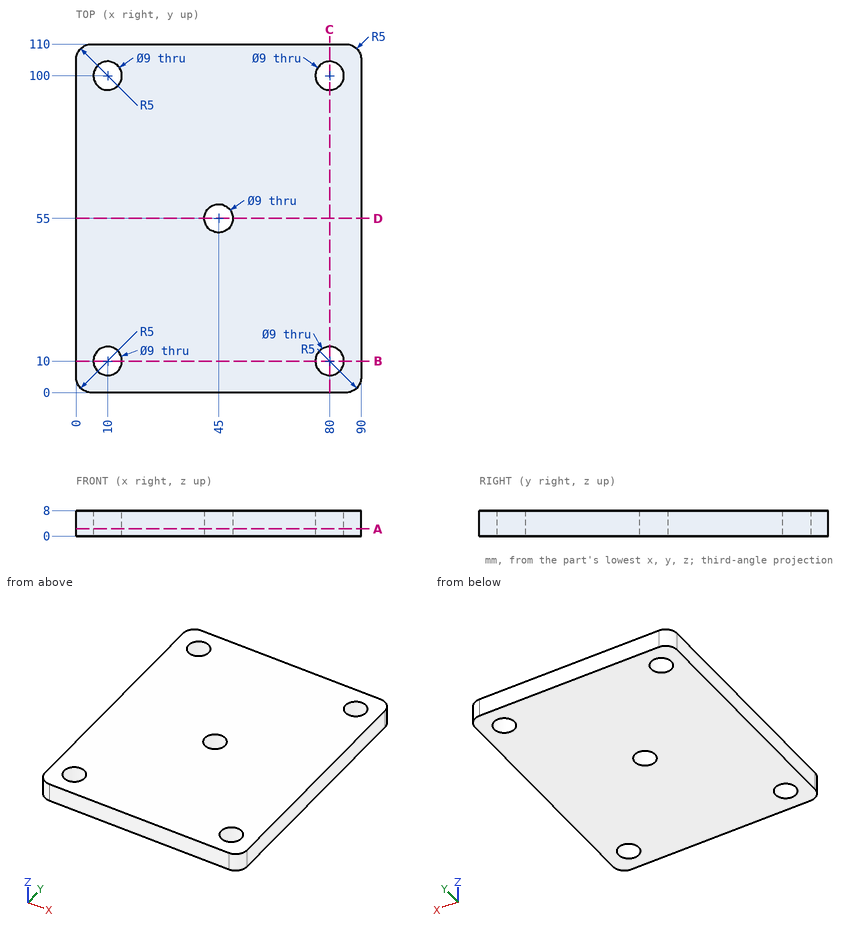
The drawing under review shows one solid part. Ordinate dimensions are in mm from its lowest x, y, z. Coordinates: 2 decimals unless noted, no trailing zeros. Order: outer loops, then holes, each group sorted by start corner. A loop starts at its lowest first (then second) coordinate and runs counter-clockwise, first axis right, second up. Notation, with made-up numbers: (55.5, 87) -> (83.5, 87) arc R16 ccw to (83.5, 101) -> close; hole circle Ø8 at (33, 15.25). An arc over 180 degrees is marked (long way). Answer in a Markdown table with one row per item.
(1) Consider section A-A (z = 2.25). Write out the cut boundary in (x, y).
Answers:
| item | result |
|---|---|
| outline | (0, 5) arc R5 ccw to (5, 0) -> (85, 0) arc R5 ccw to (90, 5) -> (90, 105) arc R5 ccw to (85, 110) -> (5, 110) arc R5 ccw to (0, 105) -> close; hole circle Ø9 at (10, 10); hole circle Ø9 at (10, 100); hole circle Ø9 at (45, 55); hole circle Ø9 at (80, 10); hole circle Ø9 at (80, 100) |
(2) Consider section C-C (x = 80). Write out the cut boundary in (y, z).
Answers:
| item | result |
|---|---|
| outline | (0, 0) -> (5.5, 0) -> (5.5, 8) -> (0, 8) -> close; (14.5, 0) -> (95.5, 0) -> (95.5, 8) -> (14.5, 8) -> close; (104.5, 0) -> (110, 0) -> (110, 8) -> (104.5, 8) -> close |
(3) Wall thickness on line 1 along Y through (x, z) = (80, 6.25); line 2 along Y through (x, z) = (45, 2); line 3 along Y through (x, z) = (81, 1.5): over which ranges is each line inside the solid? List them lowest first.
Answers:
| item | result |
|---|---|
| line 1 | 0 to 5.5, 14.5 to 95.5, 104.5 to 110 |
| line 2 | 0 to 50.5, 59.5 to 110 |
| line 3 | 0 to 5.61, 14.39 to 95.61, 104.39 to 110 |
(4) Consider section B-B (y = 10). Write out the cut boundary in (x, z), plus the area to 3 significant figures.
Answers:
| item | result |
|---|---|
| outline | (0, 0) -> (5.5, 0) -> (5.5, 8) -> (0, 8) -> close; (14.5, 0) -> (75.5, 0) -> (75.5, 8) -> (14.5, 8) -> close; (84.5, 0) -> (90, 0) -> (90, 8) -> (84.5, 8) -> close |
| area | 576 mm² |
(5) Consider section D-D (y = 55). Write out the cut boundary in (x, z).
Answers:
| item | result |
|---|---|
| outline | (0, 0) -> (40.5, 0) -> (40.5, 8) -> (0, 8) -> close; (49.5, 0) -> (90, 0) -> (90, 8) -> (49.5, 8) -> close |
(6) Insertion check: pin 1 (5 mm diameter, centred on x = 34.5, y = 30, fed in from -Z); pin 2 (7 mm diameter, centred on x = 10, y = 10, fed in from +Z). Each pin has a flat end and moves straight along its axis. Give the tip position at first contact, or say it passes through.
Answers:
| item | result |
|---|---|
| pin 1 | z = 0 |
| pin 2 | through |
